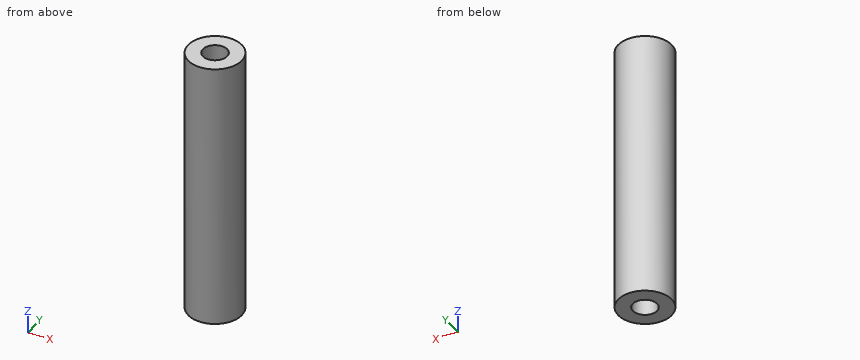
```python
from build123d import *

# Parameters (mm, degrees)
SKETCH1_R             = 7.5
BOSS_EXTRUDE1_DEPTH   = 75
M8_TAPPED_HOLE1_D     = 6.8
M8_TAPPED_HOLE1_DEPTH = 19.75
M8_TAPPED_HOLE1_TIP   = 2.042926105
M8_TAPPED_HOLE2_D     = 6.8
M8_TAPPED_HOLE2_DEPTH = 19.75
M8_TAPPED_HOLE2_TIP   = 2.042926105


with BuildPart() as part:
    # Sketch1 → Boss-Extrude1 (new body)
    with BuildSketch(Plane.XY):
        Circle(SKETCH1_R)
    extrude(amount=BOSS_EXTRUDE1_DEPTH)

    # M8 Tapped Hole1
    with Locations(Plane.XY.offset(75)):
        with Locations((0, 0)):
            Hole(M8_TAPPED_HOLE1_D / 2, depth=M8_TAPPED_HOLE1_DEPTH)
            with Locations((0, 0, -(M8_TAPPED_HOLE1_DEPTH + M8_TAPPED_HOLE1_TIP / 2))):  # 118° drill point
                Cone(0, M8_TAPPED_HOLE1_D / 2, M8_TAPPED_HOLE1_TIP, mode=Mode.SUBTRACT)

    # M8 Tapped Hole2
    with Locations(Plane(origin=(0, 0, 0), x_dir=(-1, 0, 0), z_dir=(0, 0, -1))):
        with Locations((0, 0)):
            Hole(M8_TAPPED_HOLE2_D / 2, depth=M8_TAPPED_HOLE2_DEPTH)
            with Locations((0, 0, -(M8_TAPPED_HOLE2_DEPTH + M8_TAPPED_HOLE2_TIP / 2))):  # 118° drill point
                Cone(0, M8_TAPPED_HOLE2_D / 2, M8_TAPPED_HOLE2_TIP, mode=Mode.SUBTRACT)


solid = part.part
```
Check sheet for the modelled part. Datum: model origin and axes. Units: mm. Round coordinates to 2 decimals unless told otherwise and drop trailing zeros. Write each loop counter-clockwise with the first axis right and the second up, starting at its lowest first coordinate (ties: lowest second). Pieces come first, ordered by that corner, then holes. Notation, with made-up numbers: (-20.5, 84.25) -> (23.5, 84.25) arc R29 cw to (23.5, 116.25) -> close; hole circle Ø3 at (26.25, 43). An arc over 180 degrees is marked (long way). One line per question, with ' | ' between items. Start each with the question number.
1. Sectioned sample at D-D, the plane z = 41.5. Record the cut outline in (x, y).
2. Depth check by flat-ended pin: pin 1 (2 mm diameter, centred on x = -4, z = 24.5, fed in from +Y); pin 2 (6 mm diameter, centred on x = 0, y = 0, fed in from -Z); pin 3 (2 mm diameter, centred on x = 4.5, z = 23.5, fed in from +Y). Enter the tip coordinate at first touch or a pass-through.
3. Sectioned sample at B-B, the plane y = 6. Record the cut outline in (x, z).
4. Sectioned sample at A-A, the plane z = 56.5. Record the cut outline in (x, y).
5. Scan lines: line 1 along Y through (x, z) = (0, 8.25); line 2 along Y through (x, z) = (-0.5, 54); line 3 along Y through (x, z) = (6, 18.5). Record each from-to range of solid material in increasing order. Write a range as from..to.
Taken from the geometry:
1) outline: circle Ø15 at (0, 0)
2) pin 1: stops at y = 6.87 | pin 2: stops at z = 19.99 | pin 3: stops at y = 6.63
3) outline: (-4.5, 0) -> (4.5, 0) -> (4.5, 75) -> (-4.5, 75) -> close
4) outline: circle Ø15 at (0, 0); hole circle Ø6.8 at (0, 0)
5) line 1: y = -7.5..-3.4, 3.4..7.5 | line 2: y = -7.48..-1.22, 1.22..7.48 | line 3: y = -4.5..4.5
